Part model, mm, in its own coordinate system. A direction names the side the tool comes from. Round coordinates to 2 decimals unless told otherwise and drop trailing zeros. Write each loop counter-clockwise with the first axis right and the second up, starting at its lowest first coordinate (ties: lowest second). Pieces come first, ordered by that corner, then holes. Notation, with made-up numbers: M 0.25,79 L 36.25,79 A15 cw 36.25,89 Z; hole C 59.5,88.25 d9. An arc over 180 degrees is marked long. Use one line per item in the form item = value. Start each with the question number.
Item 1: Cut at B-B, the plane x = 3. Give the cut face in (y, z), then the cut area to 3 significant figures.
Item 2: Mould opens along Y. For faces 3 (the face through (2.9, 15.6, -10.7)), 4 (the face through (0, 0, -18.9)) say: +Y half, -Y half, draft (parallel to the pull), parting line (faces both ways), or undercut.
Item 3: Probe L1, parallel to Y at x = 2, z = -20; L2, parallel to Y at x = -0.8, z = 0; L3, parallel to Y at x = -2.25, z = -7. List the from-to ranges inside material, lowest first.
Item 4: Flat gauge pins, fed straight in: pin 1 Ø5 at (y, z) = (-8, 0.5) entering from -X; pin 2 Ø0.8 at (x, y) = (-0.5, -13.5) entering from -Z; pin 3 Ø1.2 at (x, z) = (-0.5, 20.5) entering from +Y. Where does each tip first touch, or does it go through?
Item 5: Cut at D-D, the plane x = -0.25. Give the cut face in (y, z).
Item 6: Cut at C-C, the plane y = 0. Give the cut face in (x, z), then the cut area to 3 significant figures.
Item 7: Cut at A-A, the plane z = 0. Give the cut face in (x, y).
Item 8: Which spindle directions (+Z, -Z, +X, -X, +Y, -Y) get a long thin tool onto all of the face, cutting with end or side? Do faces 1 (the face through (0, 8.1, 20)), 2 (the face through (-0.03, 2.16, -6.87)). Say none if no direction does.
from build123d import *

# Parameters (mm, degrees)
EXTRUDE_1_DEPTH      = 2.1
EXTRUDE_1_DEPTH_BACK = 2.1
SKETCH_1_R           = 7.2
EXTRUDE_2_DEPTH      = 3
EXTRUDE_3_DEPTH      = 3


with BuildPart() as part:
    # 草图1 → 凸台-拉伸1 (new, two sides: drawn at the far end of the back side and taken through both)
    with BuildSketch(Plane(origin=(0, 0, 0), x_dir=(0, 0, -1), z_dir=(1, 0, 0)).offset(-EXTRUDE_1_DEPTH_BACK)):
        Polygon((-21.2, 8.1), (-18.7, 8.1), (-18.7, -8.1), (-21.2, -8.1), (-21.2, -13.569488728), (-11.5, -17.1), (21.9, -17.1), (21.9, -14.5), (19.8, -14.5), (19.8, -12), (21.9, -12), (21.9, -8.1), (18.9, -8.1), (18.9, 8.1), (21.9, 8.1), (21.9, 12), (19.8, 12), (19.8, 14.5), (21.9, 14.5), (21.9, 17.1), (-11.5, 17.1), (-21.2, 13.569488728), align=None)
        Circle(SKETCH_1_R, mode=Mode.SUBTRACT)
    extrude(amount=EXTRUDE_1_DEPTH + EXTRUDE_1_DEPTH_BACK)

    # 草图2 → 凸台-拉伸2 (add)
    with BuildSketch(Plane(origin=(0, 17.1, 0), x_dir=(1, 0, 0), z_dir=(0, 1, 0))):
        Polygon((-3.6, -10), (-2.1, -11.5), (2.1, -11.5), (3.6, -10), (3.6, 10), (2.1, 11.5), (-2.1, 11.5), (-3.6, 10), align=None)
    extrude(amount=-EXTRUDE_2_DEPTH)

    # 草图3 → 凸台-拉伸3 (add)
    with BuildSketch(Plane(origin=(0, -17.1, 0), x_dir=(1, 0, 0), z_dir=(0, 1, 0))):
        Polygon((-3.6, -10), (-2.1, -11.5), (2.1, -11.5), (3.6, -10), (3.6, 10), (2.1, 11.5), (-2.1, 11.5), (-3.6, 10), align=None)
    extrude(amount=EXTRUDE_3_DEPTH)


solid = part.part
Model answer:
q1.outline = M -17.1,-10.6 L -14.1,-10.6 L -14.1,10.6 L -17.1,10.6 Z; M 14.1,-10.6 L 17.1,-10.6 L 17.1,10.6 L 14.1,10.6 Z
q1.area = 127 mm²
q2.face_3 = draft
q2.face_4 = undercut
q3.L1 = -17.1 to -14.5, -12 to -8.1, 8.1 to 12, 14.5 to 17.1
q3.L2 = -17.1 to -7.2, 7.2 to 17.1
q3.L3 = -17.1 to -14.1, 14.1 to 17.1
q4.pin_1 = -2.1
q4.pin_2 = -19.8
q4.pin_3 = 14.04
q5.outline = M -17.1,-21.9 L -14.5,-21.9 L -14.5,-19.8 L -12,-19.8 L -12,-21.9 L -8.1,-21.9 L -8.1,-18.9 L 8.1,-18.9 L 8.1,-21.9 L 12,-21.9 L 12,-19.8 L 14.5,-19.8 L 14.5,-21.9 L 17.1,-21.9 L 17.1,11.5 L 13.57,21.2 L 8.1,21.2 L 8.1,18.7 L -8.1,18.7 L -8.1,21.2 L -13.57,21.2 L -17.1,11.5 Z; hole C 0,0 d14.4
q6.outline = M -2.1,-18.9 L 2.1,-18.9 L 2.1,-7.2 L -2.1,-7.2 Z; M -2.1,7.2 L 2.1,7.2 L 2.1,18.7 L -2.1,18.7 Z
q6.area = 97.4 mm²
q7.outline = M -3.6,-17.1 L 3.6,-17.1 L 3.6,-14.1 L 2.1,-14.1 L 2.1,-7.2 L -2.1,-7.2 L -2.1,-14.1 L -3.6,-14.1 Z; M -3.6,14.1 L -2.1,14.1 L -2.1,7.2 L 2.1,7.2 L 2.1,14.1 L 3.6,14.1 L 3.6,17.1 L -3.6,17.1 Z
q8.face_1 = +Z, +X, -X
q8.face_2 = +X, -X
